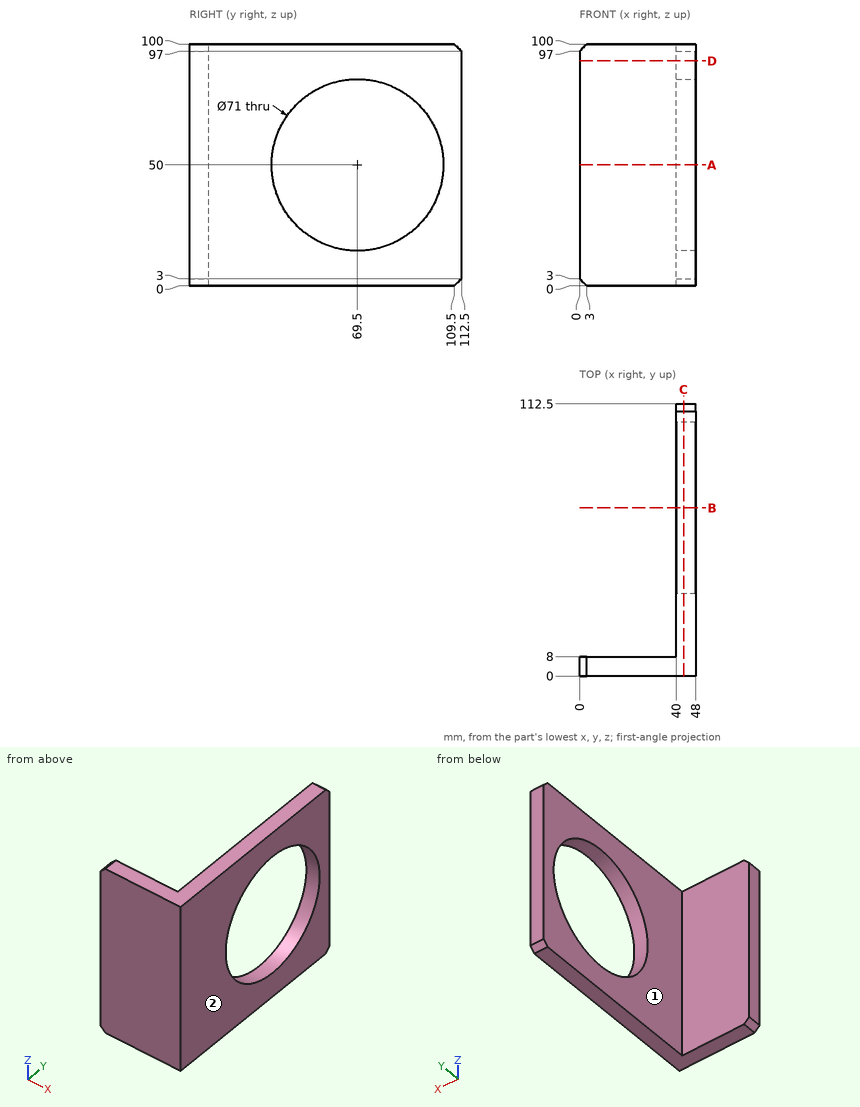
Design review of the part shown in the three views and the two pictorial views. Dimensions are in mm from the part's minimum x, y and z. A direction names the side the tool comes from. Round coordinates to 2 decimals unless told otherwise and drop trailing zeros. Write each loop counter-clockwise with the first axis right and the second up, starting at its lowest first coordinate (ties: lowest second). Pieces come first, ordered by that corner, then holes.
Item 1: Consider section C-C on x = 43. Give the boundary of the cut face in (y, z), and give its area (3 significant figures).
Item 2: Wall thickness on L1, parallel to Y at x = 42, z = 50; L2, parallel to Z at x = 43, y = 69; L3, parallel to Y at x = 11, z = 37: over which ranges is each line inside the solid? List them lowest first.
Item 3: Consider section D-D on z = 93. Give the boundary of the cut face in (x, y), and give its area (3 significant figures).
Item 4: Consider section A-A on z = 50. Give the boundary of the cut face in (x, y), and give its area (3 significant figures).
Item 5: For pin 1 Ø12 at (y, z) = (47.5, 27) entering from -X; pin 2 Ø12 at (x, z) = (15, 72.5) entering from +Y; pin 3 Ø8 at (x, y) = (13, 13) entering from +Z, all flat-tipped, find the tip position at first contact; note any pin that passes through.
Item 6: For the marked faces 1 and 2, list the 3-axis set-ups (+Z, -Z, +X, -X, +Y, -Y) from which the entire face can be reached by the end or side of a thin tool; tool diameter is ignored.
Item 7: Consider section B-B on y = 69.5. Give the boundary of the cut face in (x, z).
Check values:
1. outline: (0, 0) - (109.5, 0) - (112.5, 3) - (112.5, 97) - (109.5, 100) - (0, 100) - close; hole circle Ø71 at (69.5, 50)
1. area: 7,280 mm2
2. L1: y = 0 to 34, 105 to 112.5
2. L2: z = 0 to 14.5, 85.5 to 100
2. L3: y = 0 to 8
3. outline: (0, 0) - (48, 0) - (48, 112.5) - (40, 112.5) - (40, 8) - (0, 8) - close
3. area: 1,220 mm2
4. outline: (0, 0) - (48, 0) - (48, 34) - (40, 34) - (40, 8) - (0, 8) - close; (40, 105) - (48, 105) - (48, 112.5) - (40, 112.5) - close
4. area: 652 mm2
5. pin 1: stops at x = 40
5. pin 2: stops at y = 8
5. pin 3: passes through
6. face 1: +Z, -Z, -X, +Y
6. face 2: +Z, -Z, +X, +Y, -Y
7. outline: (40, 0) - (48, 0) - (48, 14.5) - (40, 14.5) - close; (40, 85.5) - (48, 85.5) - (48, 100) - (40, 100) - close
